```python
from build123d import *

# Parameters (mm, degrees)
SKETCH_1_R      = 6
EXTRUDE_1_DEPTH = 6
FILLET_R10_1_R  = 10


with BuildPart() as part:
    # 草图1 → 凸台-拉伸1 (new body)
    with BuildSketch(Plane.XY):
        with BuildLine():
            Line((6.614378278, 7.5), (89.385621722, 7.5))
            ThreePointArc((89.385621722, 7.5), (106, 0), (89.385621722, -7.5))
            Line((89.385621722, -7.5), (6.614378278, -7.5))
            ThreePointArc((6.614378278, -7.5), (-10, 0), (6.614378278, 7.5))
        make_face()
        Circle(SKETCH_1_R, mode=Mode.SUBTRACT)
        with Locations((96, 0)):
            Circle(SKETCH_1_R, mode=Mode.SUBTRACT)
        with BuildLine():
            Line((18, 3.5), (41, 3.5))
            ThreePointArc((41, 3.5), (44.5, 0), (41, -3.5))
            Line((41, -3.5), (18, -3.5))
            ThreePointArc((18, -3.5), (14.5, 0), (18, 3.5))
        make_face(mode=Mode.SUBTRACT)
        with BuildLine():
            Line((78, -3.5), (55, -3.5))
            ThreePointArc((55, -3.5), (51.5, 0), (55, 3.5))
            Line((55, 3.5), (78, 3.5))
            ThreePointArc((78, 3.5), (81.5, 0), (78, -3.5))
        make_face(mode=Mode.SUBTRACT)
    extrude(amount=EXTRUDE_1_DEPTH)

    # R10 圆角1
    fillet_r10_1_edges = [part.edges().sort_by_distance(p)[0] for p in [
        (6.614378278, 7.5, 3),
        (89.385621722, 7.5, 3),
        (89.385621722, -7.5, 3),
        (6.614378278, -7.5, 3),
    ]]
    fillet(fillet_r10_1_edges, radius=FILLET_R10_1_R)


solid = part.part
```
Input: part model. Units: mm. Frame: model coordinates. A direction names the side the tool comes from. Give positions to 0.01 mm unless a question says otherwise; leave off trailing zeros. Order: outer loops, then holes, each group sorted by start corner. A loop starts at its lowest first (then second) coordinate and runs counter-clockwise, first axis right, second up. Notation, with made-up numbers: (-17, 18) - (17, 18) arc R28 ccw to (17, 43) - close; hole circle Ø10 at (-8.5, -34). An arc over 180 degrees is marked (long way). Put each result on its own line as item: value.
Item 1: Access query for faces 1 (the flat face through (66, 3.5, 3)), 2 (the flat face through (49, 0, 6)). Directions: +Z, -Z, +X, -X, +Y, -Y. A direction counts if a zero-diameter tool reaches every point of the face in a straight line with its end or side. Return the directions, or none.
Found:
face 1: +Z, -Z
face 2: +Z, +X, -X, +Y, -Y
Item 2: Contact query for flat-ended pins moving along their axis: pin 1 (11 mm diameter, centred on x = 0, y = 0, fed in from +Z); pin 2 (3 mm diameter, centred on x = 51.5, z = 2, fed in from +Y); pin 3 (1 mm diameter, centred on y = 3, z = 5, fed in from -X); pin 4 (6 mm diameter, centred on x = 58.5, y = 3, fed in from +Z). Output: stop coordinate, or through.
Found:
pin 1: passes through
pin 2: stops at y = 7.5
pin 3: stops at x = -9.68
pin 4: stops at z = 6
Item 3: Section query B-B, the plane y = 0. Return loops of the section in (x, z), then the cut area to 3 significant figures.
Found:
outline: (-10, 0) - (-6, 0) - (-6, 6) - (-10, 6) - close; (6, 0) - (14.5, 0) - (14.5, 6) - (6, 6) - close; (44.5, 0) - (51.5, 0) - (51.5, 6) - (44.5, 6) - close; (81.5, 0) - (90, 0) - (90, 6) - (81.5, 6) - close; (102, 0) - (106, 0) - (106, 6) - (102, 6) - close
area: 192 mm^2
Item 4: Draft query along Y for faces 3 (the flat face through (47, 7.5, 3)), 4 (the flat face through (67, -3.5, 3)), 5 (the flat face through (49, -7.5, 3)), 6 (the cylindrical face through (81.5, 0.1, 3)). Return one class per face: +Y half, -Y half, draft (parallel to the pull), parting line (faces both ways), or undercut.
Found:
face 3: +Y half
face 4: undercut
face 5: -Y half
face 6: undercut
Item 5: Section query A-A, the plane x = 0. Return loops of the section in (y, z).
Found:
outline: (-10, 0) - (-6, 0) - (-6, 6) - (-10, 6) - close; (6, 0) - (10, 0) - (10, 6) - (6, 6) - close
Item 6: Section query C-C, the plane z = 1.7. Return loops of the section in (x, y), then the cut area to 3 significant figures.
Found:
outline: (4.84, -8.75) arc R10 cw to (9.68, -7.5) - (86.32, -7.5) arc R10 cw to (91.16, -8.75) arc R10 ccw (long way) to (91.16, 8.75) arc R10 cw to (86.32, 7.5) - (9.68, 7.5) arc R10 cw to (4.84, 8.75) arc R10 ccw (long way) to start; hole circle Ø12 at (0, 0); hole (18, -3.5) - (41, -3.5) arc R3.5 ccw to (41, 3.5) - (18, 3.5) arc R3.5 ccw to start; hole (55, -3.5) - (78, -3.5) arc R3.5 ccw to (78, 3.5) - (55, 3.5) arc R3.5 ccw to start; hole circle Ø12 at (96, 0)
area: 1,180 mm^2
Item 7: Ray query, L1, parallel to Y at x = 0, z = 2.5; L2, parallel to Y at x = 65, z = 5.05; L3, parallel to X at y = -1.5, z = 1.7. Return the intervals inside material, ascending. Write a range as from..to.
Found:
L1: y = -10..-6, 6..10
L2: y = -7.5..-3.5, 3.5..7.5
L3: x = -9.89..-5.81, 5.81..14.84, 44.16..51.84, 81.16..90.19, 101.81..105.89
